Build history of the part. All positions in model axes, mm. Face numbers are marked on the shaded views. A direction names the side the tool comes from. Coordinates: 2 decimals unless noted, no trailing zeros. Loops run counter-clockwise (first coordinate to the right, second up) from the corner with the lowest first, then second, coordinate; pieces in that order, holes last.
Item 1: Flat gauge pins, fed straight in: pin 1 (11 mm diameter, centred on y = -12.5, z = 26, fed in from +X); pin 2 (18.5 mm diameter, centred on y = -57.5, z = 53.5, fed in from -X); pin 3 (12.5 mm diameter, centred on x = 54.73, y = -61.41, fed in from +Z); pin 4 (20.5 mm diameter, centred on x = -54.73, y = -33.41, fed in from +Z). Where does each tip first touch, or does it go through?
Item 2: Cut at B-B (x = 0). List the corners of the cut face in (y, z), and give its area (3 significant figures).
Item 3: Cut at A-A (z = 29). List the corners of the cut face in (x, y), and give its area (3 significant figures).
Item 4: 3-axis set-ups, long thin cutter, end or side, ignore diameter. For the marked faces 1, 2 and 3: which of +Z, -Z, +X, -X, +Y, -Y reach the whole face in a straight line?
Item 5: Drill centre lines: line 1 along X through (y, z) = (0, 20); line 2 along Y through (x, z) = (34.5, 80); line 3 along X through (y, z) = (-67, 11). Where is each one in solid material? Low to high.
Item 6: Cut at C-C (y = -47.5). List the corners of the cut face in (x, z).
Item 7: Mould opens along X. For the marked faces 4, 5 and 6 say: released by +X, released by -X, zero draft, split by the parting line, or undercut.
Item 8: Cut at D-D (z = 46). List the corners of the cut face in (x, y), and give its area (3 significant figures).
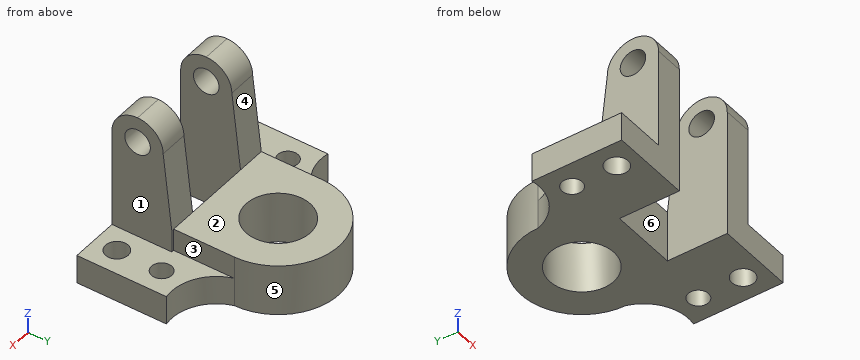
from build123d import *

# Parameters (mm, degrees)
HUB_BODY_PROFILE_R          = 20
HUB_BODY_DEPTH              = 32
MOUNTING_FLANGE_PROFILE_R   = 6.332129474
MOUNTING_FLANGE_PROFILE_R_2 = 7.040095354
MOUNTING_FLANGE_DEPTH       = 18
CLEVIS_ARMS_PROFILE_W       = 18
CLEVIS_ARMS_PROFILE_H       = 37.413354637
CLEVIS_ARMS_DEPTH           = 96
CLEVIS_SLOT_PROFILE_R       = 8
CLEVIS_SLOT_CUT_DEPTH       = 163.994398854


with BuildPart() as part:
    # Hub Body Profile → Hub Body (new body)
    with BuildSketch(Plane.XY):
        with BuildLine():
            Line((38, 0), (38, -38))
            Line((38, -38), (0, -38))
            Line((0, -38), (-38, -38))
            Line((-38, -38), (-38, 0))
            ThreePointArc((-38, 0), (0, 38), (38, 0))
        make_face()
        Circle(HUB_BODY_PROFILE_R, mode=Mode.SUBTRACT)
    extrude(amount=HUB_BODY_DEPTH)

    # Mounting Flange Profile → Mounting Flange (add)
    with BuildSketch(Plane.XY):
        with BuildLine():
            Line((-38, 0), (-38, -75.413354637))
            Line((-38, -75.413354637), (-70, -75.413354637))
            Line((-70, -75.413354637), (-70, -19.413354637))
            ThreePointArc((-70, -19.413354637), (-50.279706144, -15.839023099), (-38, 0))
        make_face()
        with Locations((-54.734551325, -33.413354637)):
            Circle(MOUNTING_FLANGE_PROFILE_R, mode=Mode.SUBTRACT)
        with Locations((-54.734551325, -61.413354637)):
            Circle(MOUNTING_FLANGE_PROFILE_R_2, mode=Mode.SUBTRACT)
    extrude(amount=MOUNTING_FLANGE_DEPTH)

    # Hub Body Mirror: part across plane


with BuildPart() as part_1:
    add(part.part)
    add(part.part.mirror(Plane(origin=(0, 0, 0), x_dir=(0, 0, 1), z_dir=(1, 0, 0))))

    # Clevis Arms Profile → Clevis Arms (add)
    with BuildSketch(Plane.XY):
        with Locations((-29, -56.706677318)):
            Rectangle(CLEVIS_ARMS_PROFILE_W, CLEVIS_ARMS_PROFILE_H)
        with Locations((30.571573125, -56.706677318)):
            Rectangle(CLEVIS_ARMS_PROFILE_W, CLEVIS_ARMS_PROFILE_H)
    extrude(amount=CLEVIS_ARMS_DEPTH)

    # Clevis Slot Profile → Clevis Slot Cut (cut, through all)
    with BuildSketch(Plane.ZY.offset(38)):
        with BuildLine():
            Line((32, -38), (80, -43.413354637))
            ThreePointArc((80, -43.413354637), (91.313708499, -48.099646138), (96, -59.413354637))
            Line((96, -59.413354637), (96, -38))
            Line((96, -38), (32, -38))
        make_face()
        with BuildLine():
            Line((96, -75.413354637), (96, -59.413354637))
            ThreePointArc((96, -59.413354637), (91.313708499, -70.727063136), (80, -75.413354637))
            Line((80, -75.413354637), (96, -75.413354637))
        make_face()
        with Locations((80, -59.413354637)):
            Circle(CLEVIS_SLOT_PROFILE_R)
    extrude(amount=-CLEVIS_SLOT_CUT_DEPTH, mode=Mode.SUBTRACT)


solid = part_1.part
Filled sheet:
1. pin 1: stops at x = 38
1. pin 2: stops at x = -38
1. pin 3: passes through
1. pin 4: stops at z = 18
2. outline: (-38, 0) - (-20, 0) - (-20, 32) - (-38, 32) - close; (20, 0) - (38, 0) - (38, 32) - (20, 32) - close
2. area: 1,150 mm2
3. outline: (-38, -75.41) - (-20, -75.41) - (-20, -38) - (21.57, -38) - (21.57, -75.41) - (39.57, -75.41) - (39.57, -38) - (38, -38) - (38, 0) arc R38 ccw to (-38, 0) - close; hole circle Ø40 at (0, 0)
3. area: 5,250 mm2
4. face 1: +Z, +X, +Y, -Y
4. face 2: +Z, +X, -X, +Y
4. face 3: +Z, +X, +Y
5. line 1: x = -38 to -20, 20 to 38
5. line 2: y = -75.41 to -67.41, -51.41 to -43.41
5. line 3: x = -70 to -59.02, -50.45 to -20, 21.57 to 50.45, 59.02 to 70
6. outline: (-70, 0) - (-20, 0) - (-20, 90.68) - (-38, 90.68) - (-38, 18) - (-70, 18) - close; (21.57, 0) - (70, 0) - (70, 18) - (39.57, 18) - (39.57, 90.68) - (21.57, 90.68) - close
7. face 4: zero draft
7. face 5: split by the parting line
7. face 6: undercut
8. outline: (-38, -75.41) - (-20, -75.41) - (-20, -39.58) - (-38, -39.58) - close; (21.57, -75.41) - (39.57, -75.41) - (39.57, -39.58) - (21.57, -39.58) - close
8. area: 1,290 mm2
